Verification items for the finished model (mm, model axes). Coordinates: 2 decimals unless noted, no trailing zeros. Loops run counter-clockwise (first coordinate to the right, second up) from the corner with the lowest first, then second, coordinate; pieces in that order, holes last. Notation, with made-up numbers: (59.5, -28.75) -> (108.5, -28.75) arc R18 cw to (108.5, -20.75) -> close; hole circle Ø7 at (76, 80). An arc over 180 degrees is marked (long way). Answer as a JSON object with one key per item and string values. Group by question number.
Q1. Scan lines: L1, parallel to Y at x = 0, z = -79; L2, parallel to Z at x = 12.5, y = -3.5; L3, parallel to X at y = 5, z = 27.5. Record each from-to range of solid material in increasing order.
Q2. Cross-section at A-A on z = -400.5. Record the boundary of the cut face in (x, y).
Q3. Gauge pin test, flat ends, axial feed: pin 1 Ø5 at (y, z) = (18, 23.5) entering from -X; pin 2 Ø8 at (x, z) = (-4, -472) entering from -Y; pin 3 Ø2 at (y, z) = (-19, -323) entering from -X. Record the tip position at first contact, or that the pin passes through.
```python
from build123d import *

# Parameters (mm, degrees)
CHAMFER1_SIZE  = 5
CHAMFER1_SIZE2 = 0.881634904
CHAMFER2_SIZE  = 1
SKETCH5_W      = 15.5
SKETCH5_H      = 1184


with BuildPart() as part:
    # Sketch3 → Revolve1 (revolve)
    with BuildSketch(Plane(origin=(0, 0, 0), x_dir=(0, 0, -1), z_dir=(1, 0, 0)), mode=Mode.PRIVATE) as revolve1_sk:
        Polygon((-300, 25), (900, 25), (900, 8.5), (905, 8.5), (905, 7.5), (920, 7.5), (920, 0), (-320, 0), (-320, 7.5), (-305, 7.5), (-305, 8.5), (-300, 8.5), align=None)
    revolve(revolve1_sk.sketch.rotate(Axis((0, 0, 320), (0, 0, -1)), 90), axis=Axis((0, 0, 320), (0, 0, -1)))

    # Chamfer1
    chamfer1_edges = [part.edges().sort_by_distance(p)[0] for p in [
        (-25, 0, -900),
        (-25, 0, 300),
    ]]
    chamfer1_side = [part.faces().sort_by_distance(p)[0] for p in [
        (-25, 0, -300),
    ]]
    chamfer(chamfer1_edges, length=CHAMFER1_SIZE, length2=CHAMFER1_SIZE2, reference=chamfer1_side[0])

    # Chamfer2
    chamfer2_edges = [part.edges().sort_by_distance(p)[0] for p in [
        (-7.5, 0, -920),
        (-7.5, 0, 320),
    ]]
    chamfer(chamfer2_edges, length=CHAMFER2_SIZE)

    # Sketch5 → Cut-Revolve1 (revolve, cut)
    with BuildSketch(Plane(origin=(0, 0, 0), x_dir=(1, 0, 0), z_dir=(0, 1, 0)), mode=Mode.PRIVATE) as cut_revolve1_sk:
        with Locations((15.25, 300)):
            Rectangle(SKETCH5_W, SKETCH5_H)
    revolve(cut_revolve1_sk.sketch.rotate(Axis((0, 0, -920), (0, 0, 1)), 180), axis=Axis((0, 0, -920), (0, 0, 1)), mode=Mode.SUBTRACT)


solid = part.part
```
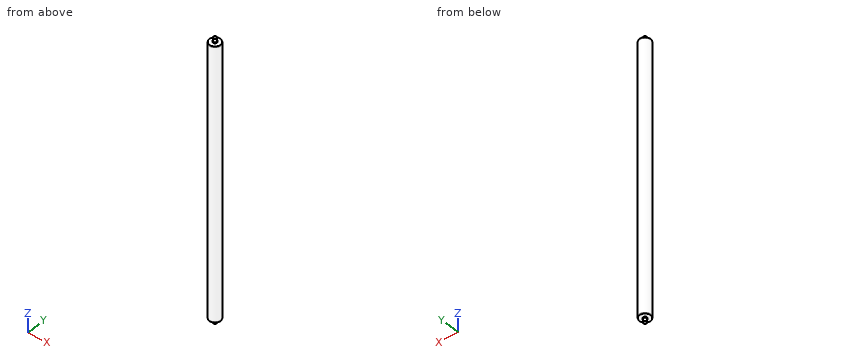
Computed values:
{
 "1": {"L1": "y = -25 to -23, -7.5 to 7.5, 23 to 25", "L2": "z = -900 to -892, 292 to 300", "L3": "x = -24.49 to -22.45, -5.59 to 5.59, 22.45 to 24.49"},
 "2": {"outline": "circle Ø50 at (0, 0); circle Ø15 at (0, 0); hole circle Ø46 at (0, 0)"},
 "3": {"pin 1": "stops at x = -19.62", "pin 2": "stops at y = -25", "pin 3": "stops at x = -17.35"}
}
